Check sheet for the modelled part. Datum: model origin and axes. Units: mm. A direction names the side the tool comes from. Round coordinates to 2 decimals unless told otherwise and drop trailing zeros. Order: outer loops, then holes, each group sorted by start corner. A loop starts at its lowest first (then second) coordinate and runs counter-clockwise, first axis right, second up.
```python
from build123d import *

# Parameters (mm, degrees)
CIRPATTERN1_COUNT   = 4
CIRPATTERN2_COUNT   = 4
BOSS_EXTRUDE1_DEPTH = 80
SHELL1_T            = -6
BOSS_EXTRUDE3_DEPTH = 6


with BuildPart() as part:
    # Sketch1 → Revolve1 (revolve)
    with BuildSketch(Plane.XY, mode=Mode.PRIVATE) as revolve1_sk:
        Polygon((-55, 0), (-72.5, 0), (-72.5, 130), (-55, 130), (-55, 99), (-49.5, 99), (-49.5, 31), (-55, 31), align=None)
    revolve(revolve1_sk.sketch.rotate(Axis((0, 0, 0), (0, 1, 0)), 270), axis=Axis((0, 0, 0), (0, 1, 0)))

    # Sketch2 → M6 Tapped Hole1 (revolve, cut)
    with BuildSketch(Plane(origin=(0, 130, -62.5), x_dir=(0, 0, 1), z_dir=(1, 0, 0))):
        Polygon((0, 0), (0, 19.502151548), (2.5, 18), (2.5, 0), align=None)
    m6_tapped_hole1 = revolve(axis=Axis((0, 136.35, -62.5), (0, -1, 0)), mode=Mode.SUBTRACT)

    # CirPattern1: M6 Tapped Hole1 ×4 about axis
    cirpattern1_axis = Axis((0, 0, 0), (0, 1, 0))
    for i in range(1, CIRPATTERN1_COUNT):
        add(m6_tapped_hole1.rotate(cirpattern1_axis, i * 360 / CIRPATTERN1_COUNT), mode=Mode.SUBTRACT)

    # Sketch4 → M6 Tapped Hole2 (revolve, cut)
    with BuildSketch(Plane(origin=(0, 0, 62.5), x_dir=(0, 0, -1), z_dir=(1, 0, 0))):
        Polygon((0, 0), (0, 19.502151548), (2.5, 18), (2.5, 0), align=None)
    m6_tapped_hole2 = revolve(axis=Axis((0, -6.35, 62.5), (0, 1, 0)), mode=Mode.SUBTRACT)

    # CirPattern2: M6 Tapped Hole2 ×4 about axis
    cirpattern2_axis = Axis((0, 0, 0), (0, 1, 0))
    for i in range(1, CIRPATTERN2_COUNT):
        add(m6_tapped_hole2.rotate(cirpattern2_axis, i * 360 / CIRPATTERN2_COUNT), mode=Mode.SUBTRACT)



with BuildPart() as body_2:
    # Sketch6 → Boss-Extrude1 (new body)
    with BuildSketch(Plane(origin=(0, 130, 0), x_dir=(1, 0, 0), z_dir=(0, 1, 0))):
        with BuildLine():
            Line((-1050, 40), (-60.466933112, 40))
            ThreePointArc((-60.466933112, 40), (-72.5, 0), (-60.466933112, -40))
            Line((-60.466933112, -40), (-1050, -40))
            Line((-1050, -40), (-1050, 40))
        make_face()
    extrude(amount=-BOSS_EXTRUDE1_DEPTH)

    # Shell1
    shell1_openings = [body_2.faces().sort_by_distance(p)[0] for p in [
        (-72.5, 90, 0),
        (-1050, 90, 0),
    ]]
    offset(amount=SHELL1_T, openings=shell1_openings, kind=Kind.INTERSECTION)


with BuildPart() as part_1:
    add(part.part)

    add(body_2.part)  # Boss-Extrude3 merges body 2
    # Sketch8 → Boss-Extrude3 (add)
    with BuildSketch(Plane.XY.offset(40)):
        Polygon((-60.466933112, 50), (-572.5, 50), (-72.5, 0), (-60.466933112, 0), align=None)
    boss_extrude3 = extrude(amount=-BOSS_EXTRUDE3_DEPTH)

    # Mirror1: Boss-Extrude3 across plane
    add(boss_extrude3.mirror(Plane.XY))


solid = part_1.part
```
Item 1: Sectioned sample at C-C (x = -211). Record the cut outline in (y, z).
Answer:
outline: (13.85, -40) - (130, -40) - (130, 40) - (13.85, 40) - (13.85, 34) - (50, 34) - (50, -34) - (13.85, -34) - close; hole (56, -34) - (124, -34) - (124, 34) - (56, 34) - close
Item 2: Sectioned sample at A-A (x = -827). Record the cut outline in (y, z).
Answer:
outline: (50, -40) - (130, -40) - (130, 40) - (50, 40) - close; hole (56, -34) - (124, -34) - (124, 34) - (56, 34) - close
Item 3: Sectioned sample at B-B (y = 88.5). Record the cut outline in (x, z), and give its area (3 significant figures).
Answer:
outline: (-1050, -40) - (-60.47, -40) arc R72.5 ccw (long way) to (-60.47, 40) - (-1050, 40) - (-1050, 34) - (-64.03, 34) arc R72.5 ccw to (-64.03, -34) - (-1050, -34) - close; hole circle Ø99 at (0, 0)
area: 20,700 mm2
Item 4: Go/stop test with flat-tipped pins: P1, Ø3, axis at x = 0, z = -62.5, coming from the -Y side; P2, Ø1, axis at x = -573.5, z = 33.5, coming from the -Y side; P3, Ø3, axis at x = 62.5, z = 0, coming from the +Y side; P4, Ø8, axis at x = -62.5, z = 0, coming from the +Y side. Record where each tip stops, or that it passes through.
Answer:
P1: stops at y = 18.6
P2: stops at y = 50
P3: stops at y = 111.4
P4: stops at y = 130
Item 5: Access from +Z, -Z, +X, -X, +Y, -Y to the whole of each face (thin tool, end or side, straight path). Record for faces 1 (the flat face through (-562, 80, -40)), 2 (the flat face through (-550, 56, 0)), 3 (the cylindrical face through (48.794, 15.283, -25.379)), 4 (the flat face through (-550, 50, -1)), 5 (the cylindrical face through (48.794, 114.283, -25.379)).
Answer:
face 1: -Z, -X, +Y, -Y
face 2: -X
face 3: -Y
face 4: -X, -Y
face 5: +Y
Item 6: Scan lines: line 1 along Z through (x, y) = (-401.5, 33.5); line 2 along X through (y, z) = (75, 0); line 3 along Y through (x, z) = (-604, -33). Record each from-to range of solid material in increasing order.
Answer:
line 1: z = -40 to -34, 34 to 40
line 2: x = -72.5 to -49.5, 49.5 to 72.5
line 3: y = 50 to 56, 124 to 130
Item 7: Release check for a two-part mould opening along Z. For faces 6 (the flat face through (-1050, 126, 1)), 7 (the cylindrical face through (-33.454, 64.524, 36.484)), 8 (the cylindrical face through (72.454, 65.91, 2.595)) record: released by +Z, released by -Z, zero draft, split by the parting line, or undercut.
Answer:
face 6: zero draft
face 7: undercut
face 8: split by the parting line
